```python
from build123d import *

# Parameters (mm, degrees)
BASE_BLOCK_PROFILE_W      = 65
BASE_BLOCK_PROFILE_H      = 25
BASE_BLOCK_65X25X50_DEPTH = 50
UPRIGHT_PROFILE_W         = 50
UPRIGHT_PROFILE_H         = 20
UPRIGHT_BLOCK_DEPTH       = 25
BOTTOM_TONGUE_PROFILE_W   = 25
BOTTOM_TONGUE_PROFILE_H   = 10
BOTTOM_TONGUE_10X25_DEPTH = 50
END_NOTCH_PROFILE_R       = 15
ROUND_END_NOTCH_DEPTH     = 50
TOP_BOSS_PROFILE_R        = 25
ROUNDED_TOP_BOSS_DEPTH    = 15
BOSS_HALF_HOLE_15_DEPTH   = 15
SUPPORT_WEDGE_DEPTH       = 50
RIB_TRIM_FRONT_DEPTH      = 20
RIB_TRIM_REAR_DEPTH       = 20


with BuildPart() as part:
    # Base Block Profile → Base Block 65x25x50 (new body)
    with BuildSketch(Plane.XY):
        with Locations((32.5, 12.5)):
            Rectangle(BASE_BLOCK_PROFILE_W, BASE_BLOCK_PROFILE_H)
    extrude(amount=-BASE_BLOCK_65X25X50_DEPTH)

    # Upright Profile → Upright Block (add)
    with BuildSketch(Plane.ZY):
        with Locations((-25, 35)):
            Rectangle(UPRIGHT_PROFILE_W, UPRIGHT_PROFILE_H)
    extrude(amount=-UPRIGHT_BLOCK_DEPTH)

    # Bottom Tongue Profile → Bottom Tongue 10x25 (add)
    with BuildSketch(Plane.XY):
        with Locations((12.5, -5)):
            Rectangle(BOTTOM_TONGUE_PROFILE_W, BOTTOM_TONGUE_PROFILE_H)
    extrude(amount=-BOTTOM_TONGUE_10X25_DEPTH)

    # End Notch Profile → Round End Notch (cut)
    with BuildSketch(Plane(origin=(0, 25, 0), x_dir=(1, 0, 0), z_dir=(0, 1, 0))):
        with Locations((65, 25)):
            Circle(END_NOTCH_PROFILE_R)
    extrude(amount=-ROUND_END_NOTCH_DEPTH, mode=Mode.SUBTRACT)

    # Top Boss Profile → Rounded Top Boss (add)
    with BuildSketch(Plane.ZY):
        with Locations((-25, 45)):
            Circle(TOP_BOSS_PROFILE_R)
    extrude(amount=-ROUNDED_TOP_BOSS_DEPTH)

    # Boss Hole Profile → Boss Half Hole Ø15 (cut)
    with BuildSketch(Plane(origin=(15, 0, 0), x_dir=(0, 0, -1), z_dir=(1, 0, 0))):
        with BuildLine():
            Line((10, 45), (40, 45))
            ThreePointArc((40, 45), (25, 60), (10, 45))
        make_face()
    extrude(amount=-BOSS_HALF_HOLE_15_DEPTH, mode=Mode.SUBTRACT)

    # Support Wedge Profile → Support Wedge (add)
    with BuildSketch(Plane.XY):
        Polygon((25, 45), (25, 25), (45, 25), align=None)
    extrude(amount=-SUPPORT_WEDGE_DEPTH)

    # Rib Trim Front Profile → Rib Trim Front (cut)
    with BuildSketch(Plane.XY):
        Polygon((25, 45), (45, 25), (25, 25), align=None)
    extrude(amount=-RIB_TRIM_FRONT_DEPTH, mode=Mode.SUBTRACT)

    # Rib Trim Rear Profile → Rib Trim Rear (cut)
    with BuildSketch(Plane(origin=(0, 0, -50), x_dir=(-1, 0, 0), z_dir=(0, 0, -1))):
        Polygon((-25, 45), (-25, 25), (-45, 25), align=None)
    extrude(amount=-RIB_TRIM_REAR_DEPTH, mode=Mode.SUBTRACT)


solid = part.part
```
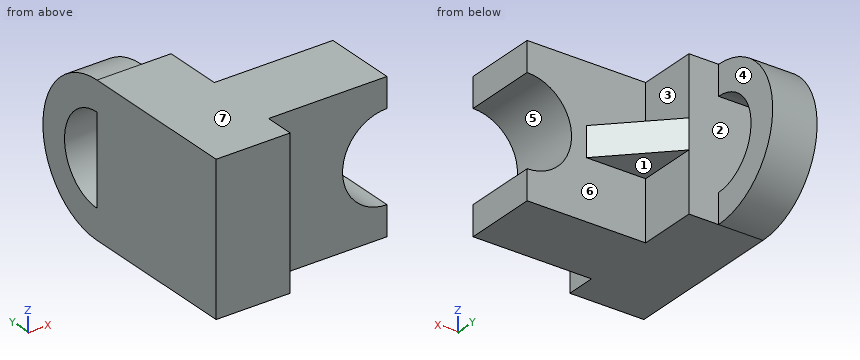
Geometry check sheet. Reference: the model listing, model coordinates, mm. Face numbers are marked on the shaded views. A direction names the side the tool comes from. Coordinates: 2 decimals unless noted, no trailing zeros. Write each loop counter-clockwise with the first axis right and the second up, starting at its lowest first coordinate (ties: lowest second). Pieces come first, ordered by that corner, then holes. Notation, with made-up numbers: (33, 28.25) -> (69, 28.25) arc R11 ccw to (69, 43.25) -> close; hole circle Ø8 at (35, 46.25). An arc over 180 degrees is marked (long way). Use CSV: the item, a comma, the result in double quotes. Start each with the question number.
Item 1: Cross-section at D-D, the plane x = 8. Record the cut outline in (y, z), plus the area to 3 significant figures.
Item 2: Set-up check for the marked faces 1, 2, 3 and 4: record each of +Z, -Z, +X, -X, +Y, -Y from which the full face is reachable in a straight line by a thin tool's end or side.
Item 3: Cross-section at A-A, the plane y = 51.5. Record the cut outline in (x, z).
Item 4: Depth check by flat-ended pin: pin 1 Ø6 at (y, z) = (34, -38) entering from +X; pin 2 Ø20 at (x, z) = (42, -18.5) entering from +Y; pin 3 Ø3 at (y, z) = (14.5, -16) entering from +X. Enter the tip coordinate at first touch or a pass-through.
Item 5: Thickness scan on line 1 (X direction, y = -2.5, z = -21); line 2 (Y direction, x = 16, z = -39.5); line 3 (X direction, y = 55, z = -41.5). Record the ranges inside material, lowest first.
Item 6: Mould release check, pull along Z, two halves, no side actions. Record for the marked faces 5, 6 and 7: released by +Z, released by -Z, zero draft, split by the parting line, or undercut.
Item 7: Cross-section at C-C, the plane x = 54. Record the cut outline in (y, z), plus the area to 3 significant figures.
Item 8: Cross-section at B-B, the plane z = -25. Record the cut outline in (x, y).
Answers:
1,outline,"(-10, -50) -> (45, -50) arc R25 ccw to (45, 0) -> (-10, 0) -> close; hole (45, -40) arc R15 ccw to (45, -10) -> close"
1,area,"3,380 mm^2"
2,face 1,"-Z, +X, +Y"
2,face 2,"+X"
2,face 3,"+Z, +X, +Y"
2,face 4,"+Z, -Z, +X, +Y"
3,outline,"(0, -49.14) -> (15, -49.14) -> (15, -38.52) -> (0, -38.52) -> close; (0, -11.48) -> (15, -11.48) -> (15, -0.86) -> (0, -0.86) -> close"
4,pin 1,"x = 25"
4,pin 2,"y = 37.89"
4,pin 3,"x = 54.29"
5,line 1,"0 to 25"
5,line 2,"-10 to 45"
5,line 3,"0 to 15"
6,face 5,"undercut"
6,face 6,"zero draft"
6,face 7,"released by +Z"
7,outline,"(0, -50) -> (25, -50) -> (25, -35.2) -> (0, -35.2) -> close; (0, -14.8) -> (25, -14.8) -> (25, 0) -> (0, 0) -> close"
7,area,"740 mm^2"
8,outline,"(0, -10) -> (25, -10) -> (25, 0) -> (50, 0) -> (50, 25) -> (45, 25) -> (25, 45) -> (0, 45) -> close; (0, 60) -> (15, 60) -> (15, 70) -> (0, 70) -> close"
